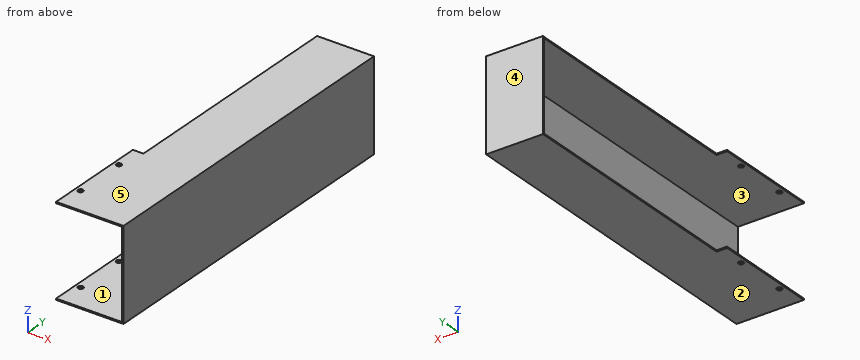
```python
from build123d import *

# Parameters (mm, degrees)
EXTRUDE_1_DEPTH        = 67
SHELL_1_T              = 1
SKETCH_2_R             = 2
CUT_EXTRUDE_1_DEPTH    = 404.809707905
PATTERN_LINEAR_1_COUNT = 2
PATTERN_LINEAR_1_PITCH = 40


with BuildPart() as part:
    # 草图1 → 凸台-拉伸1 (new body)
    with BuildSketch(Plane.XY):
        Polygon((5.123141908, -134.949925194), (5.123141908, -314.949925194), (-2.876858092, -314.949925194), (-2.876858092, -394.949925194), (47.123141908, -394.949925194), (47.123141908, -134.949925194), align=None)
    extrude(amount=EXTRUDE_1_DEPTH)

    # 抽壳1
    shell_1_openings = [part.faces().sort_by_distance(p)[0] for p in [
        (5.123141908, -224.949925194, 33.5),
        (1.123141908, -314.949925194, 33.5),
        (-2.876858092, -354.949925194, 33.5),
        (22.123141908, -394.949925194, 33.5),
    ]]
    offset(amount=SHELL_1_T, openings=shell_1_openings, kind=Kind.INTERSECTION)

    # 草图2 → 切除-拉伸1 (cut, through all)
    with BuildSketch(Plane.XY.offset(68)):
        with Locations((1.123141908, -374.949925194)):
            Circle(SKETCH_2_R)
    cut_extrude_1 = extrude(amount=-CUT_EXTRUDE_1_DEPTH, mode=Mode.SUBTRACT)

    # 阵列(线性)1: 切除-拉伸1 ×2
    with Locations(*[(0, i * PATTERN_LINEAR_1_PITCH, 0) for i in range(1, PATTERN_LINEAR_1_COUNT)]):
        add(cut_extrude_1, mode=Mode.SUBTRACT)


solid = part.part
```
Can you work these out from the model? Positions are in its coordinate system, mm. Face numbers are marked on the shaded views. A direction names the side the tool comes from. Give positions to 0.01 mm unless a question says otherwise; leave off trailing zeros. Loops run counter-clockwise (first coordinate to the right, second up) from the corner with the lowest first, then second, coordinate; pieces in that order, holes last. Notation, with made-up numbers: M -36.5,72.25 L -17.5,72.25 A26 cw -17.5,89.25 Z; hole C 21.5,-40 d6. An arc over 180 degrees is marked long. Answer in a Markdown table with one row per item.
1. If I drill on line 1 along Z through (x, y) = (33, -280.5); line 2 along Y through (x, z) = (43, 45); line 3 along X through (y, z) = (-273, 36.5), over which ranges is the centre line in solid material (lowest first)?
Taken from the geometry:
| item | result |
|---|---|
| line 1 | z = -1 to 0, 67 to 68 |
| line 2 | y = -134.95 to -133.95 |
| line 3 | x = 47.12 to 48.12 |
2. Suppose I cut it at C-C on z = 61. Write out the boundary of the cut face in (x, y), plus the area to 3 significant figures.
Taken from the geometry:
| item | result |
|---|---|
| outline | M 5.12,-134.95 L 47.12,-134.95 L 47.12,-394.95 L 48.12,-394.95 L 48.12,-133.95 L 5.12,-133.95 Z |
| area | 303 mm² |
3. For pin 1 Ø5 at (x, z) = (25.5, 40) entering from -Y; pin 2 Ø4.5 at (x, y) = (1.12, -334.95) entering from -Z; pin 3 Ø20 at (y, z) = (-317.5, 42) entering from -X; pin 4 Ø0.8 at (x, z) = (0, 67.5) entering from +Y, each with a flat end and sliding along its axis, tell me the tip position at first contact or that it passes through.
Taken from the geometry:
| item | result |
|---|---|
| pin 1 | stops at y = -134.95 |
| pin 2 | stops at z = -1 |
| pin 3 | stops at x = 47.12 |
| pin 4 | stops at y = -314.95 |
4. Suppose I cut it at A-A on y = -350.5. Write out the boundary of the cut face in (x, z).
Taken from the geometry:
| item | result |
|---|---|
| outline | M -2.88,-1 L 48.12,-1 L 48.12,68 L -2.88,68 L -2.88,67 L 47.12,67 L 47.12,0 L -2.88,0 Z |
5. Suppose I cut it at B-B on x = 44. Write out the boundary of the cut face in (y, z).
Taken from the geometry:
| item | result |
|---|---|
| outline | M -394.95,-1 L -133.95,-1 L -133.95,68 L -394.95,68 L -394.95,67 L -134.95,67 L -134.95,0 L -394.95,0 Z |
6. Thinking about a two-plate mould opening in Z: for the marked faces 3, 4 and 5, which applies, released by +Z, released by -Z, zero draft, split by the parting line, or undercut?
Taken from the geometry:
| item | result |
|---|---|
| face 3 | undercut |
| face 4 | zero draft |
| face 5 | released by +Z |
7. Which directions (+Z, -Z, +X, -X, +Y, -Y) give clear straight access to the entire face, cutting with the end or side of a thin tool? Please do the marked faces 1 and 2.
Taken from the geometry:
| item | result |
|---|---|
| face 1 | -X, -Y |
| face 2 | -Z, +X, -X, +Y, -Y |
